Check sheet for the modelled part. Datum: model origin and axes. Units: mm. A direction names the side the tool comes from. Coordinates: 2 decimals unless noted, no trailing zeros. Loops run counter-clockwise (first coordinate to the right, second up) from the corner with the lowest first, then second, coordinate; pieces in that order, holes last. Notation, with made-up numbers: M 6.5,49.25 L 56.5,49.25 A29 ccw 56.5,86.25 Z; hole C 37,32 d10. An arc over 180 degrees is marked long. Answer as CSV lines item,"result". Start each with the question number.
from build123d import *

# Parameters (mm, degrees)
SKETCH1_W                      = 70
SKETCH1_H                      = 89
SKETCH1_W_2                    = 46
SKETCH1_H_2                    = 69
BOSS_EXTRUDE1_DEPTH            = 30
FILLET2_R                      = 5
CUT_EXTRUDE1_DEPTH             = 118.136672311
M6_TAPPED_HOLE1_D              = 5
M6_TAPPED_HOLE1_DEPTH          = 15
M6_TAPPED_HOLE1_TIP            = 1.502151548
F_6_0_6_DIAMETER_HOLE1_D       = 6
F_6_0_6_DIAMETER_HOLE1_DEPTH   = 10
F_6_0_6_DIAMETER_HOLE1_TIP     = 1.802581857
F_6_5_6_5_DIAMETER_HOLE2_D     = 6.5
F_6_5_6_5_DIAMETER_HOLE2_DEPTH = 12
F_6_5_6_5_DIAMETER_HOLE2_TIP   = 1.952797012
CUT_EXTRUDE2_REACH             = 119.137
SKETCH10_W                     = 32
SKETCH10_H                     = 15
FILLET1_R                      = 5
CHAMFER1_SIZE                  = 1


with BuildPart() as part:
    # Sketch1 → Boss-Extrude1 (new, symmetric)
    with BuildSketch(Plane.XY):
        with Locations((35, 44.5)):
            Rectangle(SKETCH1_W, SKETCH1_H)
        with Locations((35, 44.5)):
            Rectangle(SKETCH1_W_2, SKETCH1_H_2, mode=Mode.SUBTRACT)
    extrude(amount=BOSS_EXTRUDE1_DEPTH, both=True)

    # Fillet2
    fillet2_edges = [part.edges().sort_by_distance(p)[0] for p in [
        (58, 10, 0),
        (58, 79, 0),
        (12, 79, 0),
        (12, 10, 0),
    ]]
    fillet(fillet2_edges, radius=FILLET2_R)

    # Sketch2 → Cut-Extrude1 (cut, through all)
    with BuildSketch(Plane.ZY):
        with BuildLine():
            Line((-12.5, 24.5), (-12.5, 64.5))
            ThreePointArc((-12.5, 64.5), (0, 77), (12.5, 64.5))
            Line((12.5, 64.5), (12.5, 24.5))
            ThreePointArc((12.5, 24.5), (0, 12), (-12.5, 24.5))
        make_face()
    extrude(amount=-CUT_EXTRUDE1_DEPTH, mode=Mode.SUBTRACT)

    # M6 Tapped Hole1
    with Locations(Plane(origin=(0, 89, 0), x_dir=(1, 0, 0), z_dir=(0, 1, 0))):
        with Locations((60, 0), (20, 20)):
            Hole(M6_TAPPED_HOLE1_D / 2, depth=M6_TAPPED_HOLE1_DEPTH)
            with Locations((0, 0, -(M6_TAPPED_HOLE1_DEPTH + M6_TAPPED_HOLE1_TIP / 2))):  # 118° drill point
                Cone(0, M6_TAPPED_HOLE1_D / 2, M6_TAPPED_HOLE1_TIP, mode=Mode.SUBTRACT)

    # Ø6.0 (6) Diameter Hole1
    with Locations(Plane(origin=(0, 89, 0), x_dir=(1, 0, 0), z_dir=(0, 1, 0))):
        with Locations((10, -11.5), (60, -11.5)):
            Hole(F_6_0_6_DIAMETER_HOLE1_D / 2, depth=F_6_0_6_DIAMETER_HOLE1_DEPTH)
            with Locations((0, 0, -(F_6_0_6_DIAMETER_HOLE1_DEPTH + F_6_0_6_DIAMETER_HOLE1_TIP / 2))):  # 118° drill point
                Cone(0, F_6_0_6_DIAMETER_HOLE1_D / 2, F_6_0_6_DIAMETER_HOLE1_TIP, mode=Mode.SUBTRACT)

    # Ø6.5 (6.5) Diameter Hole2
    with Locations(Plane(origin=(0, 0, 0), x_dir=(-1, 0, 0), z_dir=(0, -1, 0))):
        with Locations((-35, -17.5), (-35, 17.5)):
            Hole(F_6_5_6_5_DIAMETER_HOLE2_D / 2, depth=F_6_5_6_5_DIAMETER_HOLE2_DEPTH)
            with Locations((0, 0, -(F_6_5_6_5_DIAMETER_HOLE2_DEPTH + F_6_5_6_5_DIAMETER_HOLE2_TIP / 2))):  # 118° drill point
                Cone(0, F_6_5_6_5_DIAMETER_HOLE2_D / 2, F_6_5_6_5_DIAMETER_HOLE2_TIP, mode=Mode.SUBTRACT)

    # Sketch10 → Cut-Extrude2 (cut, up to next)
    with BuildSketch(Plane(origin=(0, 89, 0), x_dir=(1, 0, 0), z_dir=(0, 1, 0)), mode=Mode.PRIVATE) as cut_extrude2_sk1:
        with Locations((35, -22.5)):
            Rectangle(SKETCH10_W, SKETCH10_H)
    cut_extrude2_tool1 = extrude(cut_extrude2_sk1.sketch, amount=-CUT_EXTRUDE2_REACH, mode=Mode.PRIVATE) & part.part
    add(cut_extrude2_tool1.solids().sort_by_distance((35, 89, 22.5))[0], mode=Mode.SUBTRACT)

    # Fillet1
    fillet1_edges = [part.edges().sort_by_distance(p)[0] for p in [
        (51, 84, 15),
        (19, 84, 15),
    ]]
    fillet(fillet1_edges, radius=FILLET1_R)

    # Chamfer1
    chamfer1_edges = [part.edges().sort_by_distance(p)[0] for p in [
        (19, 84, 30),
        (51, 84, 30),
        (0, 89, 0),
        (70, 89, 0),
        (70, 0, 0),
        (0, 0, 0),
    ]]
    chamfer(chamfer1_edges, length=CHAMFER1_SIZE)


solid = part.part
Item 1: Release check for a two-part mould opening along Z. For faces 5 (the face through (19, 84, 25)), 6 (the face through (38.1, 5.07, 16.52)), 7 (the face through (20, 84, 17)) record: released by +Z, released by -Z, zero draft, split by the parting line, or undercut.
Item 2: Set-up check for faces 1 (the face through (57.69, 82.79, 0.96)), 2 (the face through (56, 78, 0)), 3 (the face through (6, 45, 12.5)), 4 (the face through (38.1, 5.07, -18.48)): record each of +Z, -Z, +X, -X, +Y, -Y from which the full face is reachable in a straight line by a thin tool's end or side.
Item 3: Sectioned sample at A-A, the plane x = 35. Record the boundary of the cut face in (y, z), and give its area (3 significant figures).
Item 4: Sectioned sample at B-B, the plane z = 0. Record the boundary of the cut face in (x, y).
Item 5: Sectioned sample at C-C, the plane y = 33.5. Record the boundary of the cut face in (x, z).
Item 6: Material ranges on line 1 (Z direction, x = 60, y = 83.5); line 2 (Z direction, x = 6, y = 42); line 3 (Y direction, x = 35, z = -6.5), recorded low to high. Write a range as from..to.
Item 7: Sectioned sample at D-D, the plane z = -16. Record the boundary of the cut face in (x, y).
Item 8: Go/stop test with a flat-tipped pin: pin 1 (3 mm diameter, centred on x = 31.5, y = 85, fed in from +Z). Record where the tip stops, or that it passes through.
Reply:
1,face 5,"zero draft"
1,face 6,"undercut"
1,face 7,"released by +Z"
2,face 1,"+Y"
2,face 2,"+Z, -Z"
2,face 3,"+X, -X"
2,face 4,"-Y"
3,outline,"M 0,-30 L 10,-30 L 10,-20.75 L 0,-20.75 Z; M 0,-14.25 L 10,-14.25 L 10,14.25 L 0,14.25 Z; M 0,20.75 L 10,20.75 L 10,30 L 0,30 Z; M 79,-30 L 89,-30 L 89,15 L 79,15 Z"
3,area,"920 mm²"
4,outline,"M 0,1 L 1,0 L 69,0 L 70,1 L 70,12 L 57,12 A5 cw 53,10 L 17,10 A5 cw 13,12 L 0,12 Z; M 0,77 L 13,77 A5 cw 17,79 L 53,79 A5 cw 57,77 L 57.5,77 L 57.5,89 L 1,89 L 0,88 Z; M 62.5,77 L 70,77 L 70,88 L 69,89 L 62.5,89 Z"
5,outline,"M 0,-30 L 12,-30 L 12,-12.5 L 0,-12.5 Z; M 0,12.5 L 12,12.5 L 12,30 L 0,30 Z; M 58,-30 L 70,-30 L 70,-12.5 L 58,-12.5 Z; M 58,12.5 L 70,12.5 L 70,30 L 58,30 Z"
6,line 1,"-30..-2.5, 2.5..8.5, 14.5..30"
6,line 2,"-30..-12.5, 12.5..30"
6,line 3,"0..10, 79..89"
7,outline,"M 0,1 L 1,0 L 32.12,0 L 32.12,10 L 17,10 A5 cw 12,15 L 12,74 A5 cw 17,79 L 53,79 A5 cw 58,74 L 58,15 A5 cw 53,10 L 37.88,10 L 37.88,0 L 69,0 L 70,1 L 70,88 L 69,89 L 1,89 L 0,88 Z"
8,pin 1,"z = 15"
